```python
from build123d import *

# Parameters (mm, degrees)
BASE_PROFILE_SKETCH_W         = 106
BASE_PROFILE_SKETCH_H         = 82
BASE_BLOCK_DEPTH              = 36
UNDERSIDE_CHANNEL_SKETCH_W    = 82
UNDERSIDE_CHANNEL_SKETCH_H    = 24
UNDERSIDE_CHANNEL_CUT_DEPTH   = 105.062481231
BASE_CORNER_FILLETS_R12_R     = 12
MOUNTING_HOLES_SKETCH_R       = 6
MOUNTING_HOLES_12_DEPTH       = 120.218287188
UPRIGHT_PLATE_SKETCH_W        = 12
UPRIGHT_PLATE_SKETCH_H        = 34
UPRIGHT_PLATE_DEPTH           = 82
SADDLE_BLOCK_DEPTH            = 70
SADDLE_GROOVE_SKETCH_R        = 10
SADDLE_GROOVE_20_DEPTH        = 82
REINFORCING_RIB_REACH         = 128.452
REINFORCING_RIB_SKETCH_WALL_W = 354.863135512
REINFORCING_RIB_SKETCH_WALL_H = 12
UPRIGHT_PLATE_FILLETS_R12_R   = 12


with BuildPart() as part:
    # Base Profile Sketch → Base Block (new body)
    with BuildSketch(Plane(origin=(0, 0, 0), x_dir=(1, 0, 0), z_dir=(0, 1, 0))):
        Rectangle(BASE_PROFILE_SKETCH_W, BASE_PROFILE_SKETCH_H)
    extrude(amount=BASE_BLOCK_DEPTH)

    # Underside Channel Sketch → Underside Channel Cut (cut, through all)
    with BuildSketch(Plane.XY.offset(41)):
        with Locations((0, 12)):
            Rectangle(UNDERSIDE_CHANNEL_SKETCH_W, UNDERSIDE_CHANNEL_SKETCH_H)
    extrude(amount=-UNDERSIDE_CHANNEL_CUT_DEPTH, mode=Mode.SUBTRACT)

    # Base Corner Fillets R12
    base_corner_fillets_r12_edges = [part.edges().sort_by_distance(p)[0] for p in [
        (47, 0, 41),
        (-47, 0, -41),
        (-47, 0, 41),
        (47, 0, -41),
    ]]
    fillet(base_corner_fillets_r12_edges, radius=BASE_CORNER_FILLETS_R12_R)

    # Mounting Holes Sketch → Mounting Holes Ø12 (cut, through all)
    with BuildSketch(Plane.ZY.offset(53)):
        with Locations((29, 12)):
            Circle(MOUNTING_HOLES_SKETCH_R)
        with Locations((-29, 12)):
            Circle(MOUNTING_HOLES_SKETCH_R)
    extrude(amount=-MOUNTING_HOLES_12_DEPTH, mode=Mode.SUBTRACT)

    # Upright Plate Sketch → Upright Plate (add)
    with BuildSketch(Plane.XY.offset(41)):
        with Locations((47, 53)):
            Rectangle(UPRIGHT_PLATE_SKETCH_W, UPRIGHT_PLATE_SKETCH_H)
    extrude(amount=-UPRIGHT_PLATE_DEPTH)

    # Saddle Block Sketch → Saddle Block (add)
    with BuildSketch(Plane.XY.offset(35)):
        with BuildLine():
            Line((53, 65), (97, 65))
            ThreePointArc((97, 65), (88.719410418, 47.801808881), (70.111111111, 43.550087053))
            ThreePointArc((70.111111111, 43.550087053), (58.269466098, 40.84444589), (53, 29.90014245))
            Line((53, 29.90014245), (53, 65))
        make_face()
    extrude(amount=-SADDLE_BLOCK_DEPTH)

    # Saddle Groove Sketch → Saddle Groove Ø20 (cut)
    with BuildSketch(Plane.XY.offset(35)):
        with Locations((75, 65)):
            Circle(SADDLE_GROOVE_SKETCH_R)
    extrude(amount=-SADDLE_GROOVE_20_DEPTH, mode=Mode.SUBTRACT)

    # Reinforcing Rib Sketch wall → Reinforcing Rib (add, up to next)
    with BuildSketch(Plane(origin=(-6, 53, 0), x_dir=(-0.940376225751, -0.340136081654, 0), z_dir=(0.340136081654, -0.940376225751, 0)), mode=Mode.PRIVATE) as reinforcing_rib_sk1:
        Rectangle(REINFORCING_RIB_SKETCH_WALL_W, REINFORCING_RIB_SKETCH_WALL_H)
    reinforcing_rib_tool1 = extrude(reinforcing_rib_sk1.sketch, amount=REINFORCING_RIB_REACH, mode=Mode.PRIVATE) - part.part
    add(reinforcing_rib_tool1.solids().sort_by_distance((-6, 53, 0))[0])

    # Upright Plate Fillets R12
    upright_plate_fillets_r12_edges = [part.edges().sort_by_distance(p)[0] for p in [
        (41, 36, 23.5),
        (41, 36, -23.5),
    ]]
    fillet(upright_plate_fillets_r12_edges, radius=UPRIGHT_PLATE_FILLETS_R12_R)


solid = part.part
```
Geometry check sheet. Reference: the model listing, model coordinates, mm. A direction names the side the tool comes from. Give positions to 0.01 mm unless a question says otherwise; leave off trailing zeros. Write each loop counter-clockwise with the first axis right and the second up, starting at its lowest first coordinate (ties: lowest second). Pieces come first, ordered by that corner, then holes.
1) Material ranges on L1, parallel to X at y = 18, z = -21; L2, parallel to Y at x = 49.5, z = -29; L3, parallel to X at y = 62, z = 19.5, recorded low to high.
2) Release check for a two-part mould opening along Y. For faces 4 (the flat face through (47, 0, 0)), 5 (the cylindrical face through (-47.08, 8.35, -33.76)), 6 (the flat face through (-5.34, 53.24, -0.08)) record: pulls with the +Y half, pulls with the -Y half, needs draft (parallel to the pull), parting line crosses it, or undercut.
3) Section check A-A, the plane x = 51. Record the boundary of the cut face in (y, z).
4) Section check D-D, the plane x = -21. Record the boundary of the cut face in (y, z), and give its area (3 significant figures).
5) Section check C-C, the plane y = 10.5. Record the boundary of the cut face in (x, z).
6) Access from +Z, -Z, +X, -X, +Y, -Y to the whole of each face (thin tool, end or side, straight path). Record for faces 1 (the flat face through (-41, 12, 1)), 2 (the flat face through (9, 47, -6)), 3 (the flat face through (70, 52, 35)).
7) Gauge pin test, flat ends, axial feed: pin 1 (1 mm diameter, centred on y = 8, z = -9.5, fed in from +X); pin 2 (17.5 mm diameter, centred on x = 67.5, y = 48.5, fed in from +Z); pin 3 (17.5 mm diameter, centred on y = 62, z = 23.5, fed in from -X); pin 4 (10 mm diameter, centred on x = -2.5, y = 61, fed in from +Z). Record the tip position at first contact, or that the pin passes through.
8) Section check B-B, the plane z = 32. Record the boundary of the cut face in (x, y), and give its area (3 significant figures).
Computed:
1. L1: x = -53 to -41, 41 to 53
1. L2: y = 0 to 6, 18 to 70
1. L3: x = 41 to 65.46, 84.54 to 96.79
2. face 4: pulls with the -Y half
2. face 5: undercut
2. face 6: pulls with the +Y half
3. outline: (0, -29) arc R12 ccw to (12, -41) - (70, -41) - (70, 41) - (12, 41) arc R12 ccw to (0, 29) - close; hole circle Ø12 at (12, -29); hole circle Ø12 at (12, 29)
4. outline: (24, -41) - (36, -41) - (36, -6) - (47.57, -6) - (47.57, 6) - (36, 6) - (36, 41) - (24, 41) - close
4. area: 1,120 mm2
5. outline: (-53, -40.91) - (-41, -40.91) - (-41, -34.81) - (-53, -34.81) - close; (-53, -23.19) - (-41, -23.19) - (-41, 23.19) - (-53, 23.19) - close; (-53, 34.81) - (-41, 34.81) - (-41, 40.91) - (-53, 40.91) - close; (41, -40.91) - (53, -40.91) - (53, -34.81) - (41, -34.81) - close; (41, -23.19) - (53, -23.19) - (53, 23.19) - (41, 23.19) - close; (41, 34.81) - (53, 34.81) - (53, 40.91) - (41, 40.91) - close
6. face 1: +Z, -Z, -Y
6. face 2: -Z, -X, +Y
6. face 3: +Z, +X, +Y, -Y
7. pin 1: stops at x = 53
7. pin 2: stops at z = 35
7. pin 3: stops at x = 41
7. pin 4: passes through
8. outline: (-53, 0.38) - (-41, 0.38) - (-41, 6.8) - (-53, 6.8) - close; (-53, 17.2) - (-41, 17.2) - (-41, 24) - (41, 24) - (41, 17.2) - (53, 17.2) - (53, 29.9) arc R14 cw to (70.11, 43.55) arc R22 ccw to (97, 65) - (85, 65) arc R10 cw to (65, 65) - (53, 65) - (53, 70) - (41, 70) - (41, 48) arc R12 cw to (29, 36) - (-53, 36) - close; (41, 0.38) - (53, 0.38) - (53, 6.8) - (41, 6.8) - close
8. area: 2,760 mm2
